Geometry check sheet. Reference: drawing and pictorial views, mm from the part's lowest x, y, z. A direction names the side the tool comes from. Coordinates: 2 decimals unless noted, no trailing zeros. Write each loop counter-clockwise with the first axis right and the second up, starting at its lowest first coordinate (ties: lowest second). Pieces come first, ordered by that corner, then holes. Notation, with made-up numbers: (-8.75, -38) - (23.25, -38) arc R10 cw to (23.25, -20) - close; hole circle Ø4 at (32, 9.25). An arc over 180 degrees is marked (long way). Use one line per item in the form item = value. Start each with the question number.
(1) Gauge pin test, flat ends, axial feed: pin 1 Ø6 at (x, z) = (14.5, 8.5) entering from -Y; pin 2 Ø1 at (x, y) = (12.5, 11) entering from +Z; pin 3 Ø1.5 at (x, z) = (10, 2) entering from +Y. Record the tip position at first contact, or that the pin passes through.
(2) Sectioned sample at C-C (x = 4). Record the cut outline in (y, z), and give its area (3 significant figures).
(3) Sectioned sample at B-B (x = 28.5). Record the cut outline in (y, z), and give its area (3 significant figures).
(4) Tool access check on the marked faces 1 and 2. Record the directions out of +Z, -Z, +X, -X, +Y, -Y that give a thin tool (end or side, any length) a straight path to the whole face; none if there is none.
(5) Material ranges on line 1 (Y direction, x = 6.5, z = 8); line 2 (X direction, y = 4.75, z = 5.75); line 3 (Y direction, x = 5, z = 4.75), recorded low to high. Write a range as [from, to].
(6) Sectioned sample at A-A (z = 5). Record the cut outline in (x, y).
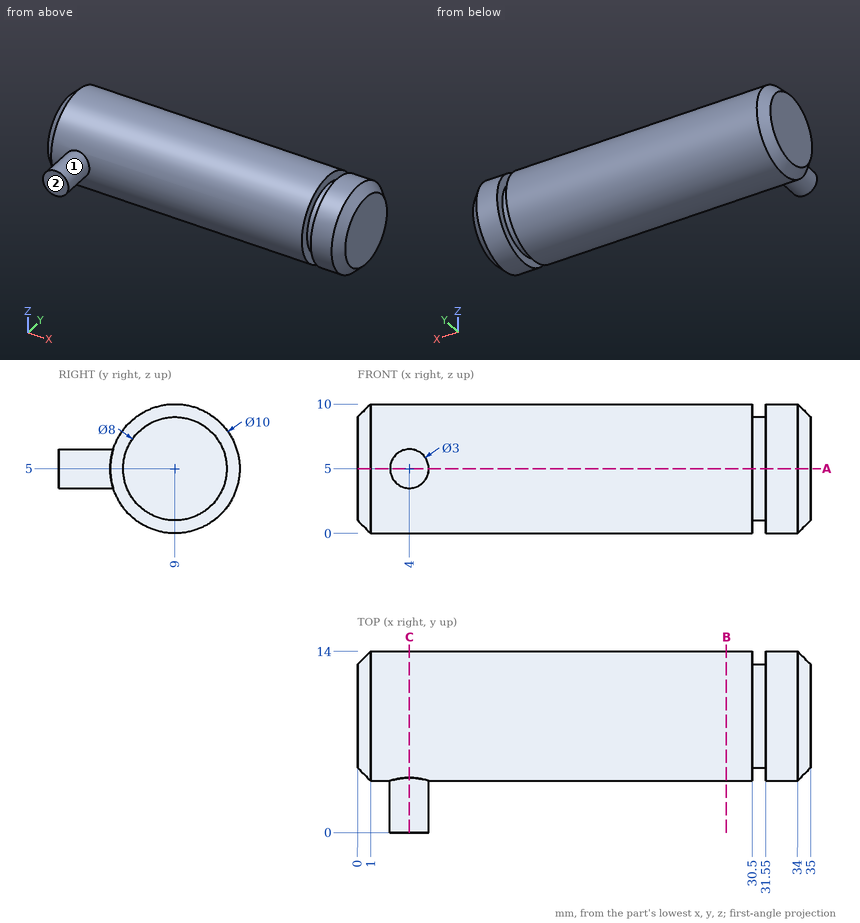
Answers below:
q1.pin_1 = 4.03
q1.pin_2 = 9.77
q1.pin_3 = 13.47
q2.outline = (0, 3.5) - (4.23, 3.5) arc R5 ccw (long way) to (4.23, 6.5) - (0, 6.5) - close
q2.area = 90.8 mm2
q3.outline = circle Ø10 at (9, 5)
q3.area = 78.5 mm2
q4.face_1 = -Y
q4.face_2 = +Z, -Z, +X, -X, -Y
q5.line_1 = [5, 13]
q5.line_2 = [0.32, 30.5], [31.55, 34.68]
q5.line_3 = [0, 13.99]
q6.outline = (0, 5) - (1, 4) - (2.5, 4) - (2.5, 0) - (5.5, 0) - (5.5, 4) - (30.5, 4) - (30.5, 5) - (31.55, 5) - (31.55, 4) - (34, 4) - (35, 5) - (35, 13) - (34, 14) - (31.55, 14) - (31.55, 13) - (30.5, 13) - (30.5, 14) - (1, 14) - (0, 13) - close
